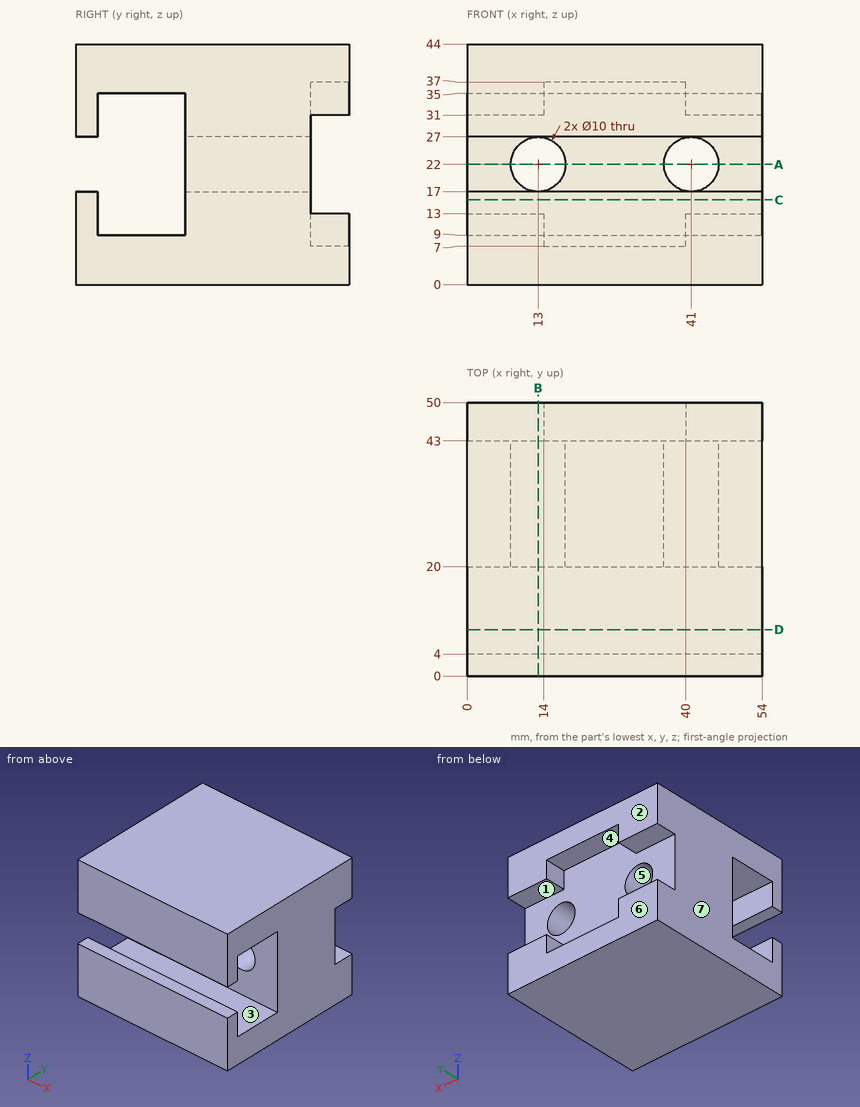
For this review, use the dimensioned drawing (mm, ordinates from the lowest corner) and the shaded views. A direction names the side the tool comes from. Round coordinates to 2 decimals unless told otherwise and drop trailing zeros. Order: outer loops, then holes, each group sorted by start corner. A loop starts at its lowest first (then second) coordinate and runs counter-clockwise, first axis right, second up. Notation, with made-up numbers: (21.25, -25) -> (59.25, -25) arc R16 ccw to (59.25, -19) -> close; hole circle Ø4 at (19, -23). An arc over 180 degrees is marked (long way). One line per item, written item: value. Start each with the question number.
Q1. Clearance check with flat-ended pins moving along their axes: pin 1 Ø9 at (x, z) = (41, 22) entering from -Y; pin 2 Ø4 at (x, z) = (29.5, 33) entering from +Y. State where each tip first meets the part, or that it passes through.
Q2. Machinability: for the marked faces 1, 2 and 3, which of the approach directions +Z, -Z, +X, -X, +Y, -Y give a long, thin tool a straight path to every point of the face, cutting with its end or side? Answer none if there is none.
Q3. Take a section at A-A (z = 22). Write out the cut boundary in (x, y), and give its area (3 significant figures).
Q4. Take a section at C-C (z = 15.5). Write out the cut boundary in (x, y), and give its area (3 significant figures).
Q5. Take a section at B-B (x = 13). Write out the cut boundary in (y, z).
Q6. Wall thickness on line 1 (X direction, y = 38.25, z = 22); line 2 (Y direction, x = 31, z = 33.5); line 3 (X direction, y = 31, z = 20.5): over which ranges is each line inside the solid? List them lowest first.
Q7. Mouldability with a two-part tool opening along X and no side actions: class the marked faces 4, 5, 6 and 7 as released by +X, released by -X, zero draft, split by the parting line, or undercut.
Q8. Take a section at D-D (y = 8.5). Write out the cut boundary in (x, z), and give its area (3 significant figures).
Reported:
1. pin 1: passes through
1. pin 2: stops at y = 43
2. face 1: +X, -X, +Y
2. face 2: +Z, -Z, +X, -X, +Y
2. face 3: +X, -X
3. outline: (0, 20) -> (8, 20) -> (8, 43) -> (0, 43) -> close; (18, 20) -> (36, 20) -> (36, 43) -> (18, 43) -> close; (46, 20) -> (54, 20) -> (54, 43) -> (46, 43) -> close
3. area: 782 mm2
4. outline: (0, 0) -> (54, 0) -> (54, 4) -> (0, 4) -> close; (0, 20) -> (54, 20) -> (54, 43) -> (0, 43) -> close
4. area: 1,460 mm2
5. outline: (0, 0) -> (50, 0) -> (50, 13) -> (43, 13) -> (43, 17) -> (20, 17) -> (20, 9) -> (4, 9) -> (4, 17) -> (0, 17) -> close; (0, 27) -> (4, 27) -> (4, 35) -> (20, 35) -> (20, 27) -> (43, 27) -> (43, 31) -> (50, 31) -> (50, 44) -> (0, 44) -> close
6. line 1: x = 0 to 8, 18 to 36, 46 to 54
6. line 2: y = 0 to 4, 20 to 43
6. line 3: x = 0 to 8.23, 17.77 to 36.23, 45.77 to 54
7. face 4: undercut
7. face 5: undercut
7. face 6: zero draft
7. face 7: released by -X
8. outline: (0, 0) -> (54, 0) -> (54, 9) -> (0, 9) -> close; (0, 35) -> (54, 35) -> (54, 44) -> (0, 44) -> close
8. area: 972 mm2
